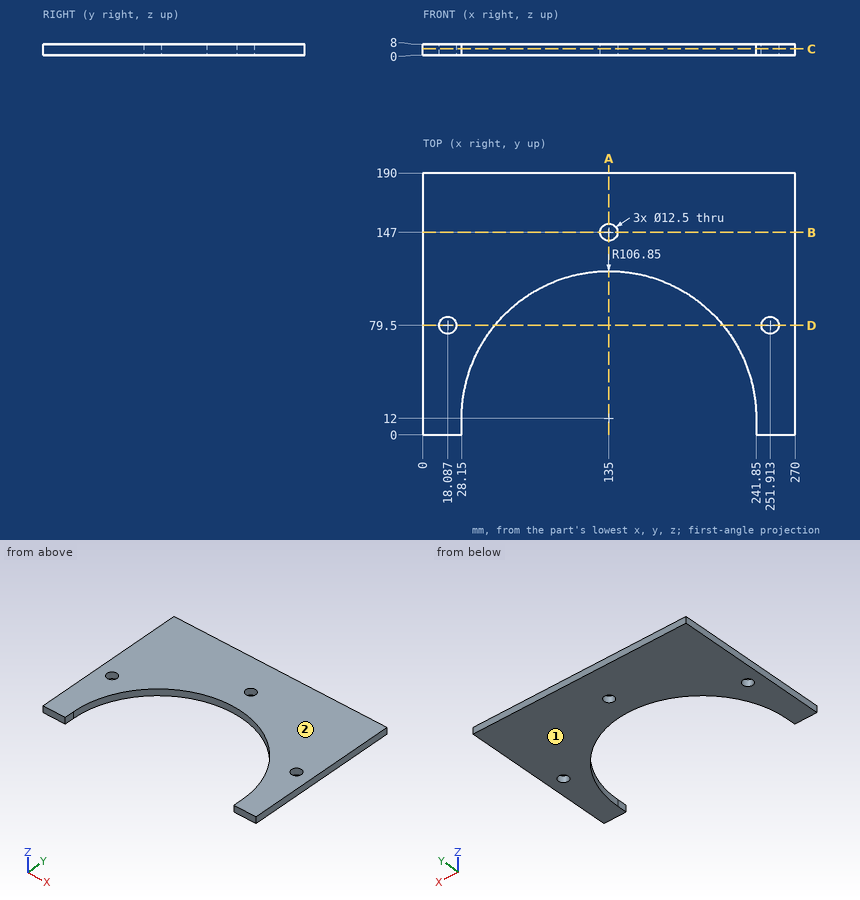
Here's the drawing with two shaded views (mm, measured from the low corner). I have some questions. Give positions to 0.01 mm unless a question says otherwise; leave off trailing zeros. Order: outer loops, then holes, each group sorted by start corner. A loop starts at its lowest first (then second) coordinate and runs counter-clockwise, first axis right, second up. Notation, with made-up numbers: M -32,51.5 L -19,51.5 A13 cw -19,75.5 Z; hole C -1.5,51 d7. An arc over 180 degrees is marked long. One line per question, with ' | ' between items.
Item 1: I'm going to push flat-ended pins straight in: pin 1 Ø2.5 at (y, z) = (7, 5.5) entering from -X; pin 2 Ø1.5 at (x, z) = (134, 6) entering from -Y. Where does each tip first touch, or does it pass through?
Answer block:
pin 1: stops at x = 0 | pin 2: stops at y = 118.84
Item 2: Suppose I cut it at D-D, the plane y = 79.5. Write out the boundary of the cut face in (x, z), then the cut area to 3 significant figures.
Answer block:
outline: M 0,0 L 11.84,0 L 11.84,8 L 0,8 Z; M 24.34,0 L 52.17,0 L 52.17,8 L 24.34,8 Z; M 217.83,0 L 245.66,0 L 245.66,8 L 217.83,8 Z; M 258.16,0 L 270,0 L 270,8 L 258.16,8 Z | area: 635 mm2
Item 3: Suppose I cut it at A-A, the plane x = 135. Write out the boundary of the cut face in (y, z).
Answer block:
outline: M 118.85,0 L 140.75,0 L 140.75,8 L 118.85,8 Z; M 153.25,0 L 190,0 L 190,8 L 153.25,8 Z
Item 4: Please list where these lines run through material, in increasing order: L1, parallel to Y at x = 135, z = 3.75; L2, parallel to Y at x = 19.5, z = 7.5; L3, parallel to X at y = 64, z = 2.75.
Answer block:
L1: y = 118.85 to 140.75, 153.25 to 190 | L2: y = 0 to 73.41, 85.59 to 190 | L3: x = 0 to 41.66, 228.34 to 270
Item 5: Suppose I cut it at B-B, the plane y = 147. Write out the boundary of the cut face in (x, z), then the cut area to 3 significant figures.
Answer block:
outline: M 0,0 L 128.75,0 L 128.75,8 L 0,8 Z; M 141.25,0 L 270,0 L 270,8 L 141.25,8 Z | area: 2,060 mm2
Item 6: Suppose I cut it at C-C, the plane z = 4.5. Write out the boundary of the cut face in (x, y).
Answer block:
outline: M 0,0 L 28.15,0 L 28.15,12 A106.85 cw 241.85,12 L 241.85,0 L 270,0 L 270,190 L 0,190 Z; hole C 18.09,79.5 d12.5; hole C 135,147 d12.5; hole C 251.91,79.5 d12.5
Item 7: We'd pull the mould along Z, two halves only. Please class the marked faces 1 and 2: released by +Z, released by -Z, zero draft, split by the parting line, or undercut.
Answer block:
face 1: released by -Z | face 2: released by +Z
